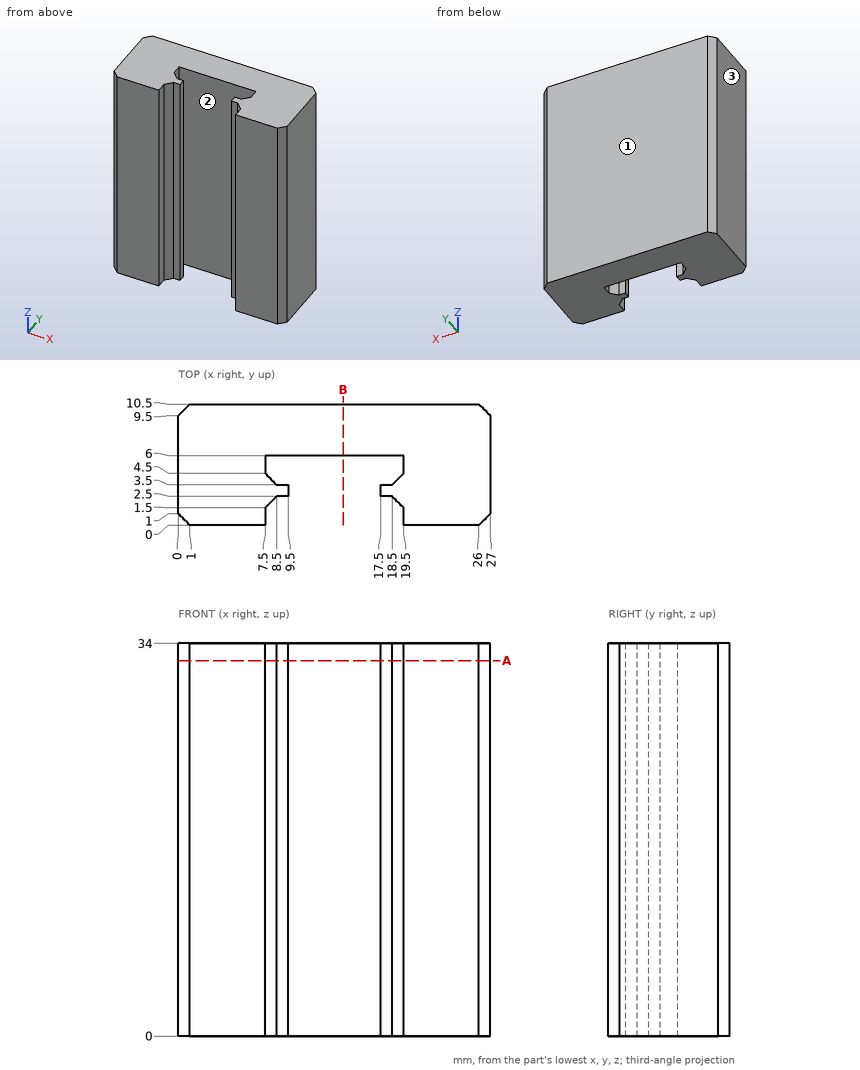
Job drawing, mm, ordinate dimensions from the low corner. One solid piece. Coordinates: 2 decimals unless noted, no trailing zeros. Loops run counter-clockwise (first coordinate to the right, second up) from the corner with the lowest first, then second, coordinate; pieces in that order, holes last. Notation, with made-up numbers: (-22, 40) - (-14, 40) arc R21 ccw to (-14, 46) - close; hole circle Ø5 at (-31, 9). An arc over 180 degrees is marked (long way). Write item = value, one per line. Start each with the question number.
Q1. Cut at B-B, the plane x = 14.25. List the corners of the cut face in (y, z).
Q2. Pull direction X, two halves, no side cores. Call the marked faces 1, 2 and 3: pulls with the +X half, pulls with the -X half, needs draft (parallel to the pull), parting line crosses it, or undercut.
Q3. Drill centre lines: L1, parallel to X at y = 5, z = 29.5; L2, parallel to Y at x = 18.25, z = 2.5; L3, parallel to Y at x = 14, z = 29. Where is each one in solid material? Low to high.
Q4. Cut at A-A, the plane z = 32.5. List the corners of the cut face in (x, y).
Q5. Flat gauge pins, fed straight in: pin 1 Ø0.5 at (x, z) = (9, 12) entering from -Y; pin 2 Ø0.8 at (y, z) = (0.5, 22) entering from -X. Where does each tip first touch, or does it go through?
Computed:
q1.outline = (6, 0) - (10.5, 0) - (10.5, 34) - (6, 34) - close
q2.face_1 = needs draft
q2.face_2 = undercut
q2.face_3 = pulls with the -X half
q3.L1 = 0 to 7.5, 19.5 to 27
q3.L2 = 2.5 to 3.5, 6 to 10.5
q3.L3 = 6 to 10.5
q4.outline = (0, 1) - (1, 0) - (7.5, 0) - (7.5, 1.5) - (8.5, 2.5) - (9.5, 2.5) - (9.5, 3.5) - (8.5, 3.5) - (7.5, 4.5) - (7.5, 6) - (19.5, 6) - (19.5, 4.5) - (18.5, 3.5) - (17.5, 3.5) - (17.5, 2.5) - (18.5, 2.5) - (19.5, 1.5) - (19.5, 0) - (26, 0) - (27, 1) - (27, 9.5) - (26, 10.5) - (1, 10.5) - (0, 9.5) - close
q5.pin_1 = 2.5
q5.pin_2 = 0.1
